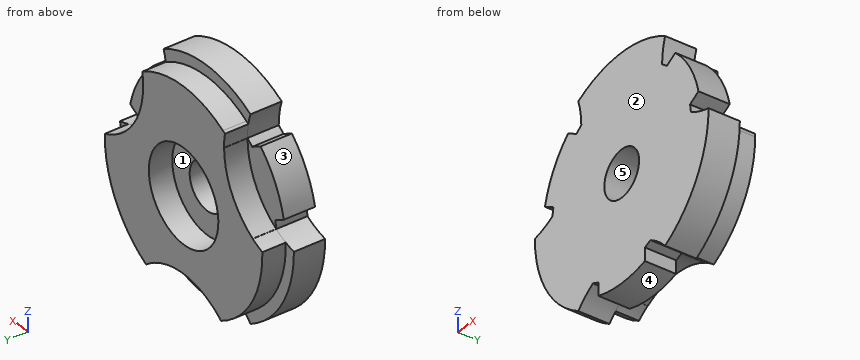
from build123d import *

# Parameters (mm, degrees)
LOBED_BASE_20MM_DEPTH          = 20
NOTCHED_START                  = -20
NOTCHED_STEP_BOSS_20MM_DEPTH   = 20
LOBED_TOP_STEP_BOSS_15MM_DEPTH = 15
COUNTERBORE_PROFILE_60_R       = 30
COUNTERBORE_60X15_DEPTH        = 15
CENTER_BORE_PROFILE_30_R       = 15
CENTER_BORE_30_DEPTH           = 60


with BuildPart() as part:
    # Lobed Base Profile → Lobed Base 20mm (new body)
    with BuildSketch(Plane(origin=(0, 0, 0), x_dir=(1, 0, 0), z_dir=(0, 1, 0))):
        with BuildLine():
            ThreePointArc((-37.5, 64.951905284), (-64.951905284, 37.5), (-75, 0))
            ThreePointArc((-75, 0), (-41.589827904, -24.011898336), (-37.5, -64.951905284))
            ThreePointArc((-37.5, -64.951905284), (0, -75), (37.5, -64.951905284))
            ThreePointArc((37.5, -64.951905284), (41.589827904, -24.011898336), (75, 0))
            ThreePointArc((75, 0), (64.951905284, 37.5), (37.5, 64.951905284))
            ThreePointArc((37.5, 64.951905284), (0, 48.023796672), (-37.5, 64.951905284))
        make_face()
    extrude(amount=LOBED_BASE_20MM_DEPTH)

    # Notched Step Profile → Notched Step Boss 20mm (add)
    with BuildSketch(Plane(origin=(0, 20, 0), x_dir=(1, 0, 0), z_dir=(0, 1, 0)).offset(NOTCHED_START)):
        with BuildLine():
            Line((66.284989118, -15.175645543), (58.989794856, -10.963763172))
            ThreePointArc((58.989794856, -10.963763172), (59.409752684, -8.395313338), (59.717932727, -5.811067957))
            ThreePointArc((59.717932727, -5.811067957), (41.589827904, -24.011898336), (34.891498837, -48.811712825))
            ThreePointArc((34.891498837, -48.811712825), (36.975430965, -47.252698388), (38.989794856, -45.604779323))
            Line((38.989794856, -45.604779323), (46.284989118, -49.816661694))
            ThreePointArc((46.284989118, -49.816661694), (58.889727457, -34), (66.284989118, -15.175645543))
        make_face()
        with BuildLine():
            Line((20, 64.992307237), (20, 56.568542495))
            ThreePointArc((20, 56.568542495), (22.434321719, 55.648011726), (24.82643389, 54.622780782))
            ThreePointArc((24.82643389, 54.622780782), (0, 48.023796672), (-24.82643389, 54.622780782))
            ThreePointArc((-24.82643389, 54.622780782), (-22.434321719, 55.648011726), (-20, 56.568542495))
            Line((-20, 56.568542495), (-20, 64.992307237))
            ThreePointArc((-20, 64.992307237), (0, 68), (20, 64.992307237))
        make_face()
        with BuildLine():
            Line((-46.284989118, -49.816661694), (-38.989794856, -45.604779323))
            ThreePointArc((-38.989794856, -45.604779323), (-36.975430965, -47.252698388), (-34.891498837, -48.811712825))
            ThreePointArc((-34.891498837, -48.811712825), (-41.589827904, -24.011898336), (-59.717932727, -5.811067957))
            ThreePointArc((-59.717932727, -5.811067957), (-59.409752684, -8.395313338), (-58.989794856, -10.963763172))
            Line((-58.989794856, -10.963763172), (-66.284989118, -15.175645543))
            ThreePointArc((-66.284989118, -15.175645543), (-58.889727457, -34), (-46.284989118, -49.816661694))
        make_face()
    extrude(amount=NOTCHED_STEP_BOSS_20MM_DEPTH)

    # Lobed Top Step Profile → Lobed Top Step Boss 15mm (add)
    with BuildSketch(Plane(origin=(0, 20, 0), x_dir=(1, 0, 0), z_dir=(0, 1, 0))):
        with BuildLine():
            ThreePointArc((-35.684614564, -57.884439044), (-34.845932731, -58.393158607), (-34, -58.889727457))
            ThreePointArc((-34, -58.889727457), (0, -68), (34, -58.889727457))
            ThreePointArc((34, -58.889727457), (34.845932731, -58.393158607), (35.684614564, -57.884439044))
            ThreePointArc((35.684614564, -57.884439044), (35.081055876, -53.366171445), (34.891498837, -48.811712825))
            ThreePointArc((34.891498837, -48.811712825), (34.925233252, -48.78758123), (34.958950977, -48.763426321))
            ThreePointArc((34.958950977, -48.763426321), (41.65016617, -24.031498852), (59.713066847, -5.860857251))
            ThreePointArc((59.713066847, -5.860857251), (59.715504976, -5.835963111), (59.717932727, -5.811067957))
            ThreePointArc((59.717932727, -5.811067957), (63.756988112, -3.697999858), (67.971701978, -1.961563214))
            ThreePointArc((67.971701978, -1.961563214), (67.992925126, -0.98088366), (68, 0))
            ThreePointArc((68, 0), (58.393158607, 34.845932731), (32.287087414, 59.846002258))
            ThreePointArc((32.287087414, 59.846002258), (28.675932236, 57.064171303), (24.82643389, 54.622780782))
            ThreePointArc((24.82643389, 54.622780782), (24.782049597, 54.642932002), (24.737648948, 54.663047157))
            ThreePointArc((24.737648948, 54.663047157), (0.01107673, 48.127580971), (-24.712484549, 54.674428277))
            ThreePointArc((-24.712484549, 54.674428277), (-24.769472681, 54.648634229), (-24.82643389, 54.622780782))
            ThreePointArc((-24.82643389, 54.622780782), (-28.675932236, 57.064171303), (-32.287087414, 59.846002258))
            ThreePointArc((-32.287087414, 59.846002258), (-58.889727457, 34), (-67.971701978, -1.961563214))
            ThreePointArc((-67.971701978, -1.961563214), (-63.756988112, -3.697999858), (-59.717932727, -5.811067957))
            ThreePointArc((-59.717932727, -5.811067957), (-59.713515872, -5.856280575), (-59.709064787, -5.901489836))
            ThreePointArc((-59.709064787, -5.901489836), (-41.66322938, -24.054276698), (-34.965372512, -48.758822023))
            ThreePointArc((-34.965372512, -48.758822023), (-34.928445686, -48.785281407), (-34.891498837, -48.811712825))
            ThreePointArc((-34.891498837, -48.811712825), (-35.081055876, -53.366171445), (-35.684614564, -57.884439044))
        make_face()
    extrude(amount=LOBED_TOP_STEP_BOSS_15MM_DEPTH)

    # Counterbore Profile Ø60 → Counterbore Ø60x15 (cut)
    with BuildSketch(Plane(origin=(0, 35, 0), x_dir=(1, 0, 0), z_dir=(0, 1, 0))):
        with Locations(Location((0, 0, 0), (0, 0, 270))):
            Circle(COUNTERBORE_PROFILE_60_R)
    extrude(amount=-COUNTERBORE_60X15_DEPTH, mode=Mode.SUBTRACT)

    # Center Bore Profile Ø30 → Center Bore Ø30 (cut)
    with BuildSketch(Plane(origin=(0, 20, 0), x_dir=(1, 0, 0), z_dir=(0, 1, 0))):
        with Locations(Location((0, 0, 0), (0, 0, 270))):
            Circle(CENTER_BORE_PROFILE_30_R)
    extrude(amount=-CENTER_BORE_30_DEPTH, mode=Mode.SUBTRACT)


solid = part.part
Geometry: final body of the model. Coordinates: model frame, mm. Face numbers are marked on the shaded views. A direction names the side the tool comes from. Round coordinates to 2 decimals unless told otherwise and drop trailing zeros. Loops run counter-clockwise (first coordinate to the right, second up) from the corner with the lowest first, then second, coordinate; pieces in that order, holes last. Notation, with made-up numbers: (6.5, 54) - (63.5, 54) arc R13 ccw to (63.5, 66) - close; hole circle Ø10 at (60, 79.5). An arc over 180 degrees is marked (long way). Write each question's results on one line, items separated by ' | '. Start each with the question number.
1) Mould query, pull axis Z, two halves, no side actions, for the marked faces 3, 4 and 5. Classes: released by +Z, released by -Z, zero draft, split by the parting line, or undercut.
2) Line query: probe 1 along Z at (x, y) = (1, 6.5); probe 2 along X at (y, z) = (22.5, -10); probe 3 along X at (y, z) = (6, 47.5). Output: solid intervals per line, ascending. Write a range as [from, to].
3) Cut plane C-C on z = 40. Return loops of the section in (x, y), then the cut area to 3 significant figures.
4) Cut plane D-D on y = 29.5. Return loops of the section in (x, z).
5) Cut plane B-B on y = 16.5. Return loops of the section in (x, z), then the cut area to 3 significant figures.
6) First-contact query: P1, Ø4, axis at x = -38.5, y = 17, coming from the -Z side; P2, Ø6, axis at x = 33.5, y = 9.5, coming from the -Z side; P3, Ø16, axis at x = -8.5, z = -60.5, coming from the +Y side. Flat tips, straight axial feed; report the tip coordinate or a pass-through.
7) Cut plane A-A on x = 0. Return loops of the section in (y, z), then the cut area to 3 significant figures.
8) Access query for the marked faces 1 and 2. Directions: +Z, -Z, +X, -X, +Y, -Y. A direction counts if a zero-diameter tool reaches every point of the face in a straight line with its end or side. Return the directions, or none.
Verdict:
1) face 3: released by +Z | face 4: released by -Z | face 5: undercut
2) probe 1: z = [-67.99, -14.97], [14.97, 74.99] | probe 2: x = [-67.26, -28.28], [28.28, 67.26] | probe 3: x = [-48.66, -42.27], [-36.66, 36.66], [42.27, 48.66]
3) outline: (-54.99, 0) - (54.99, 0) - (54.99, 20) - (35.78, 20) - (35.78, 35) - (-35.79, 35) - (-35.79, 20) - (-54.99, 20) - close | area: 3,270 mm2
4) outline: (-67.97, 1.96) arc R68 ccw to (-32.29, -59.85) arc R50 cw to (-24.83, -54.62) arc R60 ccw to (-24.71, -54.67) arc R50 cw to (24.74, -54.66) arc R60 ccw to (24.83, -54.62) arc R50 cw to (32.29, -59.85) arc R68 ccw to (68, 0) arc R68 ccw to (67.97, 1.96) arc R50 cw to (59.72, 5.81) arc R60 ccw to (59.71, 5.86) arc R50 cw to (34.96, 48.76) arc R60 ccw to (34.89, 48.81) arc R50 cw to (35.68, 57.88) arc R68 ccw to (-35.68, 57.88) arc R50 cw to (-34.89, 48.81) arc R60 ccw to (-34.97, 48.76) arc R50 cw to (-59.71, 5.9) arc R60 ccw to (-59.72, 5.81) arc R50 cw to start; hole circle Ø60 at (0, 0)
5) outline: (-75, 0) arc R75 ccw to (-37.5, -64.95) arc R50 cw to (-24.83, -54.62) arc R60 ccw to (-20, -56.57) - (-20, -64.99) arc R68 ccw to (20, -64.99) - (20, -56.57) arc R60 ccw to (24.83, -54.62) arc R50 cw to (37.5, -64.95) arc R75 ccw to (75, 0) arc R50 cw to (59.72, 5.81) arc R60 ccw to (58.99, 10.96) - (66.28, 15.18) arc R68 ccw to (46.28, 49.82) - (38.99, 45.6) arc R60 ccw to (34.89, 48.81) arc R50 cw to (37.5, 64.95) arc R75 ccw to (-37.5, 64.95) arc R50 cw to (-34.89, 48.81) arc R60 ccw to (-38.99, 45.6) - (-46.28, 49.82) arc R68 ccw to (-66.28, 15.18) - (-58.99, 10.96) arc R60 ccw to (-59.72, 5.81) arc R50 cw to start; hole circle Ø30 at (0, 0) | area: 15,000 mm2
6) P1: stops at z = -64.95 | P2: stops at z = -63.85 | P3: stops at y = 20
7) outline: (0, -68) - (20, -68) - (20, -48.13) - (35, -48.13) - (35, -30) - (20, -30) - (20, -15) - (0, -15) - close; (0, 15) - (20, 15) - (20, 30) - (35, 30) - (35, 68) - (20, 68) - (20, 75) - (0, 75) - close | area: 3,100 mm2
8) face 1: +Y | face 2: +Z, -Z, +X, -X, -Y
